Geometry: final body of the model. Coordinates: model frame, mm. A direction names the side the tool comes from. Coordinates: 2 decimals unless noted, no trailing zeros. Loops run counter-clockwise (first coordinate to the right, second up) from the corner with the lowest first, then second, coordinate; pieces in that order, holes last. Notation, with made-up numbers: (-38.5, -17.5) -> (-21.5, -17.5) arc R8 cw to (-21.5, -8.5) -> close; hole circle Ø11 at (63.25, 48.5). An arc over 180 degrees is marked (long way). One line per item, written item: value. Start each with the question number.
Item 1: Set-up query: faces 1 (the cylindrical face through (29.719, 29.594, 1.652)), 2 (the cylindrical face through (26.859, 26.797, 1.652)). Return all of +Z, -Z, +X, -X, +Y, -Y with unobstructed straight access to the full face (end or side cutting, diameter ignored); none if empty.
Item 2: Section query A-A on y = 1. Return loops of the section in (x, z).
Item 3: Ray query, probe 1 along Y at (x, z) = (-19, -90); probe 2 along X at (y, z) = (27.5, -5.5). Return the intervals inside material, ascending. Write a range as from..to.
Item 4: Mould query, pull axis X, two halves, no side actions, for faces 3 (the cylindrical face through (-29.594, 29.719, 1.652)), 4 (the cylindrical face through (29.594, -29.719, 1.652)), 5 (the cylindrical face through (-26.859, -26.797, 1.652)). Classes: +X half, -X half, draft (parallel to the pull), parting line (faces both ways), or undercut.
Item 5: Section query C-C on z = -56.5. Return loops of the section in (x, y).
Item 6: Contact query for a flat-ended pin moving along its axis: pin 1 Ø12 at (x, y) = (18.5, 2.5) entering from -Z. Output: stop coordinate, or through.
from build123d import *

# Parameters (mm, degrees)
BOSS_EXTRUDE_1_DEPTH = 118


with BuildPart() as part:
    # Sketch 1 → Boss-Extrude 1 (new, symmetric)
    with BuildSketch(Plane.XY):
        with BuildLine():
            Line((0, 32), (-24, 32))
            ThreePointArc((-24, 32), (-29.656854249, 29.656854249), (-32, 24))
            Line((-32, 24), (-32, 0))
            Line((-32, 0), (-32, -24))
            ThreePointArc((-32, -24), (-29.656854249, -29.656854249), (-24, -32))
            Line((-24, -32), (24, -32))
            ThreePointArc((24, -32), (29.656854249, -29.656854249), (32, -24))
            Line((32, -24), (32, 0))
            Line((32, 0), (32, 24))
            ThreePointArc((32, 24), (29.656854249, 29.656854249), (24, 32))
            Line((24, 32), (0, 32))
        make_face()
        with BuildLine():
            Line((0, 28), (-24, 28))
            ThreePointArc((-24, 28), (-26.828427125, 26.828427125), (-28, 24))
            Line((-28, 24), (-28, 0))
            Line((-28, 0), (-28, -24))
            ThreePointArc((-28, -24), (-26.828427125, -26.828427125), (-24, -28))
            Line((-24, -28), (24, -28))
            ThreePointArc((24, -28), (26.828427125, -26.828427125), (28, -24))
            Line((28, -24), (28, 0))
            Line((28, 0), (28, 24))
            ThreePointArc((28, 24), (26.828427125, 26.828427125), (24, 28))
            Line((24, 28), (0, 28))
        make_face(mode=Mode.SUBTRACT)
    extrude(amount=BOSS_EXTRUDE_1_DEPTH, both=True)


solid = part.part
Reply:
1. face 1: +Z, -Z, +X, +Y
1. face 2: +Z, -Z
2. outline: (-32, -118) -> (-28, -118) -> (-28, 118) -> (-32, 118) -> close; (28, -118) -> (32, -118) -> (32, 118) -> (28, 118) -> close
3. probe 1: y = -32..-28, 28..32
3. probe 2: x = -31.19..-25.94, 25.94..31.19
4. face 3: -X half
4. face 4: +X half
4. face 5: undercut
5. outline: (-32, -24) arc R8 ccw to (-24, -32) -> (24, -32) arc R8 ccw to (32, -24) -> (32, 24) arc R8 ccw to (24, 32) -> (-24, 32) arc R8 ccw to (-32, 24) -> close; hole (-28, -24) arc R4 ccw to (-24, -28) -> (24, -28) arc R4 ccw to (28, -24) -> (28, 24) arc R4 ccw to (24, 28) -> (-24, 28) arc R4 ccw to (-28, 24) -> close
6. pin 1: passes through
